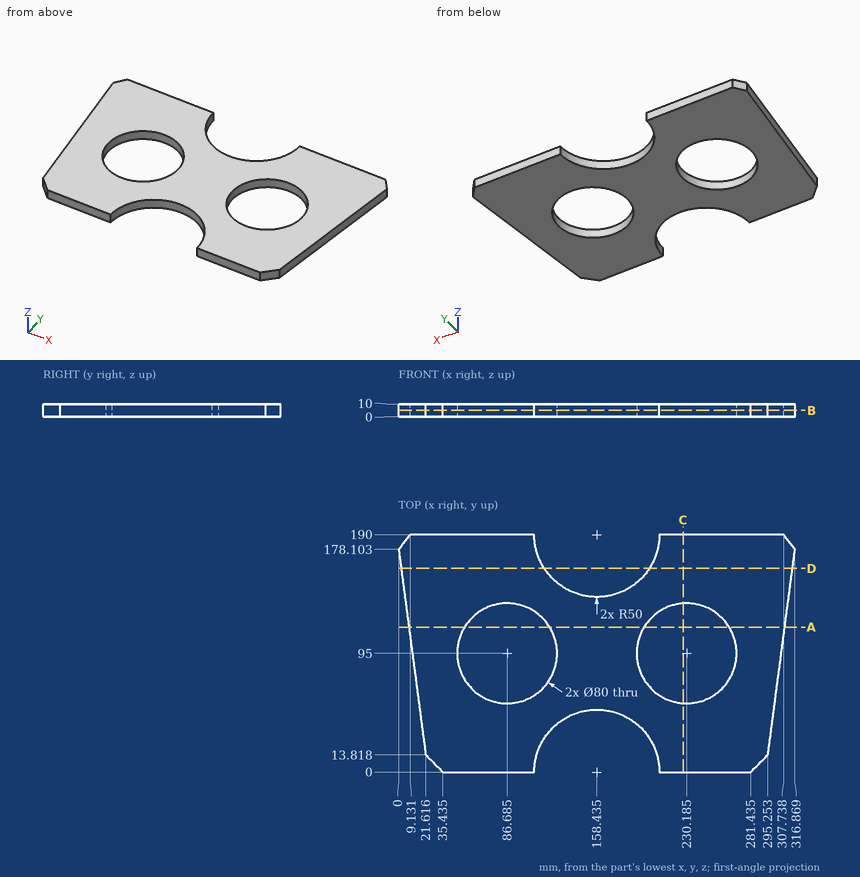
Answer from the drawing. Dimensions are ordinates in mm from the lowest x, y and z of the part. Coordinates: 2 decimals unless noted, no trailing zeros. Loops run counter-clockwise (first coordinate to the right, second up) from the corner with the lowest first, then second, coordinate; pieces in that order, holes last. Notation, with made-up numbers: (-13, 63) - (-9, 63) arc R26 ccw to (-9, 95) - close; hole circle Ø10 at (24.25, -31.75). An arc over 180 degrees is marked (long way). Use a Markdown table: item, result.
Item 1: Find section C-C, the plane x = 227.5. Determine the outline of the cut face in (y, z), and give its area (3 significant figures).
Evaluation:
| item | result |
|---|---|
| outline | (0, 0) - (55.09, 0) - (55.09, 10) - (0, 10) - close; (134.91, 0) - (190, 0) - (190, 10) - (134.91, 10) - close |
| area | 1,100 mm2 |
Item 2: Find section A-A, the plane y = 116. Determine the outline of the cut face in (x, z).
Evaluation:
| item | result |
|---|---|
| outline | (8.17, 0) - (52.64, 0) - (52.64, 10) - (8.17, 10) - close; (120.73, 0) - (196.14, 0) - (196.14, 10) - (120.73, 10) - close; (264.23, 0) - (308.7, 0) - (308.7, 10) - (264.23, 10) - close |
Item 3: Consider probe 1 along X at (y, z) = (116, 2.25); probe 2 along Y at (x, z) = (117.5, 8) (1 decimal); probe 3 along X at (y, z) = (169, 7.25). Determine where each line is inside the solid, lowest interval first. Write a range as from..to.
Evaluation:
| item | result |
|---|---|
| probe 1 | x = 8.17..52.64, 120.73..196.14, 264.23..308.7 |
| probe 2 | y = 28.7..69.5, 120.5..161.3 |
| probe 3 | x = 1.2..113.06, 203.81..315.67 |
Item 4: Find section B-B, the plane z = 5. Determine the outline of the cut face in (x, y) (1 decimal).
Evaluation:
| item | result |
|---|---|
| outline | (0, 178.1) - (21.6, 13.8) - (35.4, 0) - (108.4, 0) arc R50 cw to (208.4, 0) - (281.4, 0) - (295.3, 13.8) - (316.9, 178.1) - (307.7, 190) - (208.4, 190) arc R50 cw to (108.4, 190) - (9.1, 190) - close; hole circle Ø80 at (86.7, 95); hole circle Ø80 at (230.2, 95) |
Item 5: Find section D-D, the plane y = 163. Determine the outline of the cut face in (x, z), and give its area (3 significant figures).
Evaluation:
| item | result |
|---|---|
| outline | (1.99, 0) - (116.35, 0) - (116.35, 10) - (1.99, 10) - close; (200.52, 0) - (314.88, 0) - (314.88, 10) - (200.52, 10) - close |
| area | 2,290 mm2 |
Item 6: Given pin 1 Ø6 at (x, z) = (120, 4) entering from -Y (1 decimal); pin 2 Ø2 at (y, z) = (112.5, 2) entering from -X; pin 3 Ø1 at (y, z) = (44.5, 8.5) entering from -X; pin 4 Ø12 at (x, y) = (145, 37) entering from +Z, each flat-ended and moving along its own axis, determine where each tip first touches the part or whether it passes through.
Evaluation:
| item | result |
|---|---|
| pin 1 | stops at y = 28 |
| pin 2 | stops at x = 8.5 |
| pin 3 | stops at x = 17.51 |
| pin 4 | passes through |
